```python
from build123d import *

# Parameters (mm, degrees)
BOSS_EXTRUDE1_DEPTH         = 350
CHAMFER1_SIZE               = 3
SKETCH2_W                   = 75
SKETCH2_H                   = 230
CUT_EXTRUDE1_DEPTH          = 395.884460879
FILLET1_R                   = 10
HOLE1_D                     = 9
HOLE1_DEPTH                 = 17
HOLE1_CBORE_D               = 15
HOLE1_CBORE_DEPTH           = 10.5
M4_TAPPED_HOLE1_D           = 3.3
M4_TAPPED_HOLE1_CSINK_D     = 4.05
M4_TAPPED_HOLE1_CSINK_ANGLE = 90
HOLE2_D                     = 31
HOLE2_DEPTH                 = 3
HOLE3_D                     = 30
HOLE3_DEPTH                 = 3
M8_TAPPED_HOLE1_D           = 6.8
M6_TAPPED_HOLE2_D           = 5


with BuildPart() as part:
    # Sketch1 → Boss-Extrude1 (new body)
    with BuildSketch(Plane.XY):
        Polygon((16.751856783, 37.381546135), (146.751856783, 37.381546135), (146.751856783, 40.381546135), (168.751856783, 40.381546135), (168.751856783, 37.381546135), (181.751856783, 37.381546135), (181.751856783, 57.381546135), (-98.248143217, 57.381546135), (-98.248143217, 37.381546135), (-5.248143217, 37.381546135), (-5.248143217, 40.381546135), (16.751856783, 40.381546135), align=None)
    extrude(amount=BOSS_EXTRUDE1_DEPTH)

    # Chamfer1
    chamfer1_edges = [part.edges().sort_by_distance(p)[0] for p in [
        (181.751856783, 47.381546135, 0),
        (-98.248143217, 47.381546135, 0),
        (181.751856783, 47.381546135, 350),
        (-98.248143217, 47.381546135, 350),
    ]]
    chamfer(chamfer1_edges, length=CHAMFER1_SIZE)

    # Sketch2 → Cut-Extrude1 (cut, through all)
    with BuildSketch(Plane.XZ.offset(-37.381546135)):
        with Locations((84.251856783, 175)):
            Rectangle(SKETCH2_W, SKETCH2_H)
    extrude(amount=-CUT_EXTRUDE1_DEPTH, mode=Mode.SUBTRACT)

    # Fillet1
    fillet1_edges = [part.edges().sort_by_distance(p)[0] for p in [
        (46.751856783, 47.381546135, 60),
        (46.751856783, 47.381546135, 290),
        (121.751856783, 47.381546135, 290),
        (121.751856783, 47.381546135, 60),
    ]]
    fillet(fillet1_edges, radius=FILLET1_R)

    # Hole1
    with Locations(Plane(origin=(0, 37.381546135, 0), x_dir=(-1, 0, 0), z_dir=(0, -1, 0))):
        with Locations((38.248143217, -310), (-136.751856783, -310), (-136.751856783, -40), (38.248143217, -40)):
            CounterBoreHole(HOLE1_D / 2, HOLE1_CBORE_D / 2, HOLE1_CBORE_DEPTH, depth=HOLE1_DEPTH)

    # M4 Tapped Hole1 (through all)
    with Locations(Plane(origin=(0, 40.381546135, 0), x_dir=(-1, 0, 0), z_dir=(0, -1, 0))):
        with Locations((-5.751856783, -290), (-5.751856783, -230), (-5.751856783, -170), (-157.751856783, -170), (-157.751856783, -230), (-157.751856783, -290), (-5.751856783, -110), (-157.751856783, -110)):
            CounterSinkHole(M4_TAPPED_HOLE1_D / 2, M4_TAPPED_HOLE1_CSINK_D / 2, counter_sink_angle=M4_TAPPED_HOLE1_CSINK_ANGLE)

    # Hole2
    with Locations(Plane(origin=(0, 57.381546135, 0), x_dir=(1, 0, 0), z_dir=(0, 1, 0))):
        with Locations((-38.248143217, -310), (136.751856783, -40)):
            Hole(HOLE2_D / 2, depth=HOLE2_DEPTH)

    # Hole3
    with Locations(Plane(origin=(0, 57.381546135, 0), x_dir=(1, 0, 0), z_dir=(0, 1, 0))):
        with Locations((-38.248143217, -40), (136.751856783, -310)):
            Hole(HOLE3_D / 2, depth=HOLE3_DEPTH)

    # M8 Tapped Hole1 (through all)
    with Locations(Plane(origin=(0, 57.381546135, 0), x_dir=(1, 0, 0), z_dir=(0, 1, 0))):
        with Locations((96.751856783, -315), (66.751856783, -315), (96.751856783, -35), (66.751856783, -35)):
            Hole(M8_TAPPED_HOLE1_D / 2)

    # M6 Tapped Hole2 (through all)
    with Locations(Plane(origin=(0, 57.381546135, 0), x_dir=(1, 0, 0), z_dir=(0, 1, 0))):
        with Locations((-58.248143217, -80), (-58.248143217, -55), (-88.248143217, -55), (-88.248143217, -80)):
            Hole(M6_TAPPED_HOLE2_D / 2)


solid = part.part
```
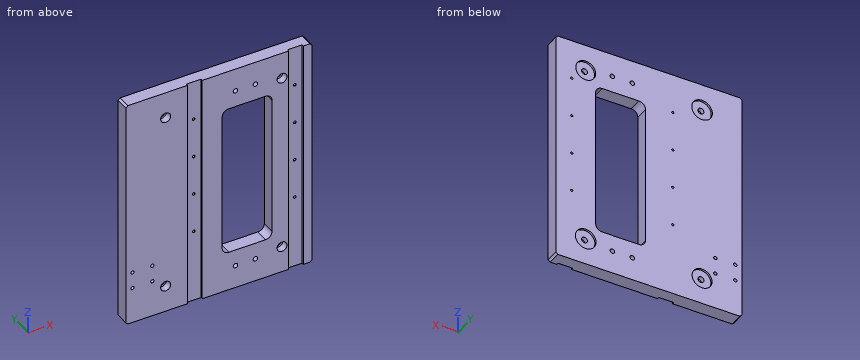
Here's how the part is built. I have some questions about the finished solid (model axes, mm). Round coordinates to 2 decimals unless told otherwise and drop trailing zeros. Order: outer loops, then holes, each group sorted by start corner. A loop starts at its lowest first (then second) coordinate and runs counter-clockwise, first axis right, second up. Notation, with made-up numbers: (-28, 59.25) -> (13, 59.25) arc R16 ccw to (13, 81.25) -> close; hole circle Ø2 at (61.5, 19). An arc over 180 degrees is marked (long way). Use a Markdown table: item, result. Add a question column.
(1) I need wall thicknesses on line 1 along X through (y, z) = (38.5, 131); line 2 along X through (y, z) = (55.75, 39.5); line 3 along X through (y, z) = (51.5, 310). Which ranges of each line are inside material? Lowest first, please.
(2) For pin 1 Ø11 at (x, z) = (66.75, 35) entering from -Y; pin 2 Ø10.5 at (x, z) = (136.75, 310) entering from +Y; pin 3 Ø11 at (x, z) = (155, 246) entering from -Y; pin 4 Ø4 at (x, z) = (-58.25, 55) entering from -Y, each with a flat end and sliding along its axis, tell me the tip position at first contact or that it passes through.
(3) Suppose I cut it at B-B, the plane z = 216.5. Please give me the cut outline in (x, y).
(4) Suppose I cut it at A-A, the plane x = 106.5. Please give me the cut outline in (y, z), and give its area (3 significant figures).
Verdict:
| question | item | result |
|---|---|---|
| 1 | line 1 | -98.25 to -5.25, 16.75 to 46.75, 121.75 to 146.75, 168.75 to 181.75 |
| 1 | line 2 | -98.25 to -53.24, -23.26 to 121.26, 152.24 to 181.75 |
| 1 | line 3 | -98.25 to -42.75, -33.75 to 132.25, 141.25 to 181.75 |
| 2 | pin 1 | y = 37.38 |
| 2 | pin 2 | y = 54.38 |
| 2 | pin 3 | y = 40.38 |
| 2 | pin 4 | through |
| 3 | outline | (-98.25, 37.38) -> (-5.25, 37.38) -> (-5.25, 40.38) -> (16.75, 40.38) -> (16.75, 37.38) -> (46.75, 37.38) -> (46.75, 57.38) -> (-98.25, 57.38) -> close; (121.75, 37.38) -> (146.75, 37.38) -> (146.75, 40.38) -> (168.75, 40.38) -> (168.75, 37.38) -> (181.75, 37.38) -> (181.75, 57.38) -> (121.75, 57.38) -> close |
| 4 | outline | (37.38, 0) -> (57.38, 0) -> (57.38, 60) -> (37.38, 60) -> close; (37.38, 290) -> (57.38, 290) -> (57.38, 350) -> (37.38, 350) -> close |
| 4 | area | 2,400 mm2 |
